from build123d import *

# Parameters (mm, degrees)
SKETCH_1_W             = 80
SKETCH_1_H             = 70
EXTRUDE_1_DEPTH        = 10
HOLE_WIZARD_M5_1_D     = 4.2
HOLE_WIZARD_M5_1_DEPTH = 14
HOLE_WIZARD_M5_1_TIP   = 1.2618073
HOLE_WIZARD_M5_2_D     = 4.2
HOLE_WIZARD_M5_2_DEPTH = 14
HOLE_WIZARD_M5_2_TIP   = 1.2618073


with BuildPart() as part:
    # 草图1 → 凸台-拉伸1 (new body)
    with BuildSketch(Plane.XY):
        Rectangle(SKETCH_1_W, SKETCH_1_H)
    extrude(amount=EXTRUDE_1_DEPTH)

    # M5 螺纹孔1
    with Locations(Plane(origin=(40, 0, 0), x_dir=(0, 0, -1), z_dir=(1, 0, 0))):
        with Locations((-5, -25), (-5, 25)):
            Hole(HOLE_WIZARD_M5_1_D / 2, depth=HOLE_WIZARD_M5_1_DEPTH)
            with Locations((0, 0, -(HOLE_WIZARD_M5_1_DEPTH + HOLE_WIZARD_M5_1_TIP / 2))):  # 118° drill point
                Cone(0, HOLE_WIZARD_M5_1_D / 2, HOLE_WIZARD_M5_1_TIP, mode=Mode.SUBTRACT)

    # M5 螺纹孔2
    with Locations(Plane.ZY.offset(40)):
        with Locations((5, 25), (5, -25)):
            Hole(HOLE_WIZARD_M5_2_D / 2, depth=HOLE_WIZARD_M5_2_DEPTH)
            with Locations((0, 0, -(HOLE_WIZARD_M5_2_DEPTH + HOLE_WIZARD_M5_2_TIP / 2))):  # 118° drill point
                Cone(0, HOLE_WIZARD_M5_2_D / 2, HOLE_WIZARD_M5_2_TIP, mode=Mode.SUBTRACT)


solid = part.part
Could you check a few things on this model? Use its own coordinates, in mm. A direction names the side the tool comes from. Give positions to 0.01 mm unless a question says otherwise; leave off trailing zeros. Order: outer loops, then holes, each group sorted by start corner. A loop starts at its lowest first (then second) coordinate and runs counter-clockwise, first axis right, second up. Notation, with made-up numbers: (57, 14) - (113, 14) arc R36 ccw to (113, 50) - close; hole circle Ø2 at (-28, 17). An arc over 180 degrees is marked (long way). Return JSON: item names as keys, results as strings. Group by question number.
Q1. Thinking about a two-plate mould opening in Z: for faces 1 (the face through (-1, 0, 0)), 2 (the face through (-1, 0, 10)), 3 (the face through (40, 0, 5)), 4 (the face through (-32.9, 26.77, 3.87)), which applies, pulls with the +Z half, pulls with the -Z half, needs draft (parallel to the pull), parting line crosses it, or undercut?
Q2. Will these pins go through, and if not, where does the flat tip stop? pin 1 Ø3.5 at (y, z) = (25, 5) entering from +X; pin 2 Ø4 at (y, z) = (25, 5) entering from +X.
Q3. Suppose I cut it at A-A, the plane x = -33.5. Please give me the cut outline in (y, z), and give its area (3 significant figures).
Q4. Please list where these lines run through material, in increasing order: line 1 along Y through (x, z) = (-35.5, 5); line 2 along Z through (x, y) = (-36, -25); line 3 along Y through (x, z) = (-28, 6.5). Write a range as [from, to].
Q5. Which directions (+Z, -Z, +X, -X, +Y, -Y) give clear straight access to the entire face, cutting with the end or side of a thin tool? Please do faces 5 (the face through (-32.9, -23.23, 3.87)), 6 (the face through (-1, 35, 5)), 7 (the face through (32.9, 26.77, 6.13)).
Resolved:
{
 "1": {"face 1": "pulls with the -Z half", "face 2": "pulls with the +Z half", "face 3": "needs draft", "face 4": "undercut"},
 "2": {"pin 1": "stops at x = 25.79", "pin 2": "stops at x = 25.94"},
 "3": {"outline": "(-35, 0) - (35, 0) - (35, 10) - (-35, 10) - close; hole circle Ø4.2 at (-25, 5); hole circle Ø4.2 at (25, 5)", "area": "672 mm2"},
 "4": {"line 1": "y = [-35, -27.1], [-22.9, 22.9], [27.1, 35]", "line 2": "z = [0, 2.9], [7.1, 10]", "line 3": "y = [-35, -26.47], [-23.53, 23.53], [26.47, 35]"},
 "5": {"face 5": "-X", "face 6": "+Z, -Z, +X, -X, +Y", "face 7": "+X"}
}
